The listing builds one solid part. Answer for the finished solid, in the listing's coordinates (mm). A direction names the side the tool comes from. Give positions to 0.01 mm unless a question says otherwise; leave off trailing zeros. Order: outer loops, then holes, each group sorted by start corner. A loop starts at its lowest first (then second) coordinate and runs counter-clockwise, first axis right, second up. Notation, with made-up numbers: (37, 41) - (43, 41) arc R21 cw to (43, 47) - close; hole circle Ø3 at (-16, 48). An arc over 180 degrees is marked (long way). Use CSV: the item, a comma, the result in double quotes.
```python
from build123d import *

# Parameters (mm, degrees)
SKETCH_1_W             = 291
SKETCH_1_H             = 134
EXTRUDE_1_DEPTH        = 6
CUT_EXTRUDE_1_DEPTH    = 161.633900532
HOLE_WIZARD_M6_1_D     = 5
HOLE_WIZARD_M6_1_DEPTH = 15
HOLE_WIZARD_M6_1_TIP   = 1.502151548
HOLE_WIZARD_M6_2_D     = 5
HOLE_WIZARD_M6_2_DEPTH = 15
HOLE_WIZARD_M6_2_TIP   = 1.502151548


with BuildPart() as part:
    # 草图1 → 凸台-拉伸1 (new, symmetric)
    with BuildSketch(Plane(origin=(0, 0, 0), x_dir=(1, 0, 0), z_dir=(0, 1, 0))):
        Rectangle(SKETCH_1_W, SKETCH_1_H)
    extrude(amount=EXTRUDE_1_DEPTH, both=True)

    # 草图2 → 切除-拉伸1 (cut, through all)
    with BuildSketch(Plane(origin=(0, 6, 0), x_dir=(1, 0, 0), z_dir=(0, 1, 0))):
        Polygon((-145.5, -67), (125.5, -67), (-145.5, 47), align=None)
        with BuildLine():
            Line((115.5, -15.191630897), (115.5, 27))
            ThreePointArc((115.5, 27), (112.571067812, 34.071067812), (105.5, 37))
            Line((105.5, 37), (5.202351114, 37))
            ThreePointArc((5.202351114, 37), (-4.600106168, 28.977834985), (1.324822524, 17.782366246))
            Line((1.324822524, 17.782366246), (101.62247141, -24.409264651))
            ThreePointArc((101.62247141, -24.409264651), (111.032843487, -23.521555443), (115.5, -15.191630897))
        make_face()
    extrude(amount=-CUT_EXTRUDE_1_DEPTH, mode=Mode.SUBTRACT)

    # M6 螺纹孔1
    with Locations(Plane(origin=(145.5, 0, 0), x_dir=(0, 0, -1), z_dir=(1, 0, 0))):
        with Locations((-57, 0), (43, 0)):
            Hole(HOLE_WIZARD_M6_1_D / 2, depth=HOLE_WIZARD_M6_1_DEPTH)
            with Locations((0, 0, -(HOLE_WIZARD_M6_1_DEPTH + HOLE_WIZARD_M6_1_TIP / 2))):  # 118° drill point
                Cone(0, HOLE_WIZARD_M6_1_D / 2, HOLE_WIZARD_M6_1_TIP, mode=Mode.SUBTRACT)

    # M6 螺纹孔2
    with Locations(Plane(origin=(0, 0, -67), x_dir=(-1, 0, 0), z_dir=(0, 0, -1))):
        with Locations((135.5, 0), (25.5, 0), (-84.5, 0)):
            Hole(HOLE_WIZARD_M6_2_D / 2, depth=HOLE_WIZARD_M6_2_DEPTH)
            with Locations((0, 0, -(HOLE_WIZARD_M6_2_DEPTH + HOLE_WIZARD_M6_2_TIP / 2))):  # 118° drill point
                Cone(0, HOLE_WIZARD_M6_2_D / 2, HOLE_WIZARD_M6_2_TIP, mode=Mode.SUBTRACT)


solid = part.part
```
Item 1: The part is cut by section B-B (x = 96.5). Give the vertices of the cut face in (y, z).
Taken from the geometry:
outline,"(-6, -67) - (6, -67) - (6, -37) - (-6, -37) - close; (-6, 22.25) - (6, 22.25) - (6, 54.8) - (-6, 54.8) - close"
Item 2: Which of the six approach directions +Z, -Z, +X, -X, +Y, -Y give full straight-line access (tool end or side, diameter ignored) to faces 1 (the face through (82, 0, -59)), 2 (the face through (137.9, -0.96, -40.69)), 3 (the face through (135, 0, 67)), 4 (the face through (112.65, 0.08, -33.99))?
Taken from the geometry:
face 1,"-Z"
face 2,"+X"
face 3,"+Z, +X, -X, +Y, -Y"
face 4,"+Y, -Y"
Item 3: The mould has two halves that part along Y. Classify faces 5 (the face through (-4.56, 0.08, -29.17)), 6 (the face through (-25.9, -0.17, -50.76)), 7 (the face through (30, -6, -1)): +Y half, -Y half, draft (parallel to the pull), parting line (faces both ways), or undercut.
Taken from the geometry:
face 5,"draft"
face 6,"undercut"
face 7,"-Y half"
Item 4: The part is cut by section A-A (z = -10). Give the vertices of the cut face in (x, y) (3 decimals).
Taken from the geometry:
outline,"(-57.544, -6) - (19.825, -6) - (19.825, 6) - (-57.544, 6) - close; (115.5, -6) - (145.5, -6) - (145.5, 6) - (115.5, 6) - close"
Item 5: Find the intervals of material crossed by line 1 along Z through (x, y) = (135, 0); line 2 along X through (y, z) = (0, -56.75); line 3 along Y through (x, z) = (136.5, -43), in increasing order.
Taken from the geometry:
line 1,"-67 to -45.5, -40.5 to 54.5, 59.5 to 67"
line 2,"-145.5 to -138, -133 to -28, -23 to 82, 87 to 145.5"
line 3,"-6 to -2.5, 2.5 to 6"
Item 6: Each of these flat-tipped pins is pushed along its axis until it touches: pin 1 (3 mm diameter, centred on y = 0, z = -43, fed in from -X); pin 2 (4.5 mm diameter, centred on x = 84.5, y = 0, fed in from -Z); pin 3 (3.5 mm diameter, centred on x = 31.5, y = 0.5, fed in from +Z). Where does it stop, or does it pass through?
Taken from the geometry:
pin 1,"x = -139.56"
pin 2,"z = -51.85"
pin 3,"z = 28.19"
Item 7: The part is cut by section C-C (x = -84). Give the vertices of the cut face in (y, z).
Taken from the geometry:
outline,"(-6, -67) - (6, -67) - (6, -21.13) - (-6, -21.13) - close"
Item 8: The part is cut by section D-D (x = -42). Give the vertices of the cut face in (y, z), and give its area (3 significant figures).
Taken from the geometry:
outline,"(-6, -67) - (6, -67) - (6, -3.46) - (-6, -3.46) - close"
area,"762 mm^2"
